Here's the drawing with two shaded views (mm, measured from the low corner). I have some questions. Coordinates: 2 decimals unless noted, no trailing zeros. Write each loop counter-clockwise with the first axis right and the second up, starting at its lowest first coordinate (ties: lowest second). Pieces come first, ordered by that corner, then holes.
Item 1: I'm going to push a flat-ended pin straight in: pin 1 Ø2 at (x, y) = (679, 32.5) entering from -Z. Where does the tip first touch, or does it pass through?
Item 2: If we section it at A-A (x = 303): Please give me the cut outline in (y, z).
Item 3: If we section it at B-B (z = 16.5): Please give me the cut outline in (x, y), then the cut area to 3 significant figures.
Item 4: If we section it at C-C (y = 82): Please give me the cut outline in (x, z).
Item 5: If I drill on line 1 (X direction, y = 131, z = 7.25); line 2 (X direction, y = 98, z = 5.5); line 3 (Y direction, x = 297, z = 11), over which ranges is the centre line in solid material (lowest first)?
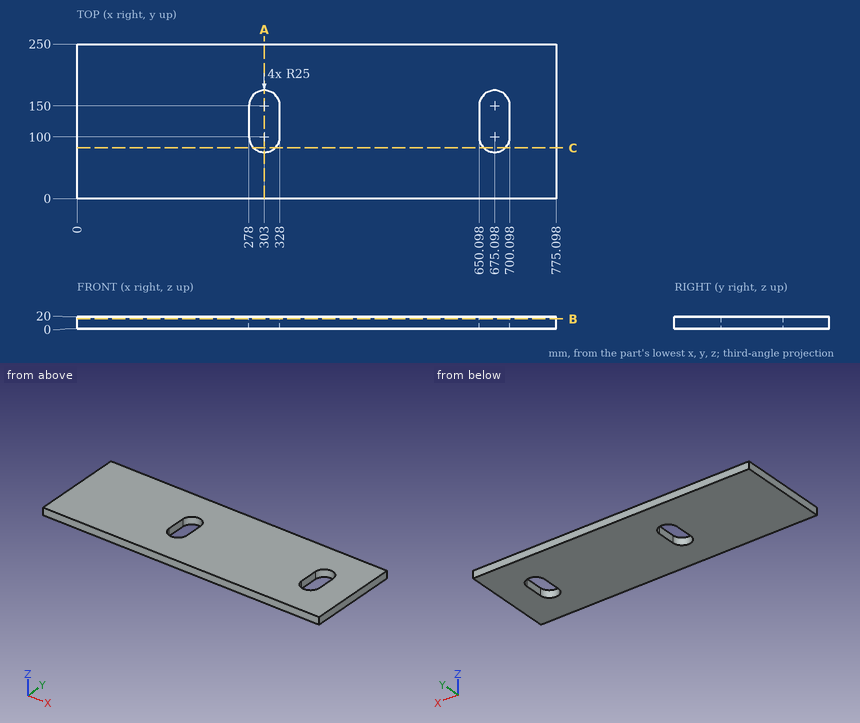
Answer list:
1. pin 1: stops at z = 0
2. outline: (0, 0) - (75, 0) - (75, 20) - (0, 20) - close; (175, 0) - (250, 0) - (250, 20) - (175, 20) - close
3. outline: (0, 0) - (775.1, 0) - (775.1, 250) - (0, 250) - close; hole (278, 100) arc R25 ccw to (328, 100) - (328, 150) arc R25 ccw to (278, 150) - close; hole (650.1, 100) arc R25 ccw to (700.1, 100) - (700.1, 150) arc R25 ccw to (650.1, 150) - close
3. area: 185,000 mm2
4. outline: (0, 0) - (285.65, 0) - (285.65, 20) - (0, 20) - close; (320.35, 0) - (657.75, 0) - (657.75, 20) - (320.35, 20) - close; (692.45, 0) - (775.1, 0) - (775.1, 20) - (692.45, 20) - close
5. line 1: x = 0 to 278, 328 to 650.1, 700.1 to 775.1
5. line 2: x = 0 to 278.08, 327.92 to 650.18, 700.02 to 775.1
5. line 3: y = 0 to 75.73, 174.27 to 250
